```python
from build123d import *

# Parameters (mm, degrees)
SKETCH_1_W              = 510
SKETCH_1_H              = 510
EXTRUDE_1_DEPTH         = 12.5
HOLE_WIZARD_10_0_10_2_D = 10
HOLE_WIZARD_15_0_15_1_D = 15
HOLE_WIZARD_M8_1_D      = 6.8
CHAMFER_1_SIZE          = 20


with BuildPart() as part:
    # 草图1 → 凸台-拉伸1 (new, symmetric)
    with BuildSketch(Plane(origin=(0, 0, 0), x_dir=(1, 0, 0), z_dir=(0, 1, 0))):
        Rectangle(SKETCH_1_W, SKETCH_1_H)
    extrude(amount=EXTRUDE_1_DEPTH, both=True)

    # Ø10.0 (10) 直径孔2 (through all)
    with Locations(Plane(origin=(0, -12.5, 0), x_dir=(-1, 0, 0), z_dir=(0, -1, 0))):
        with Locations((188, -185), (188, -140), (-188, -185), (-188, -140), (170, 203), (125, 203), (-125, 203), (-170, 203)):
            Hole(HOLE_WIZARD_10_0_10_2_D / 2)

    # Ø15.0 (15) 直径孔1 (through all)
    with Locations(Plane(origin=(0, 12.5, 0), x_dir=(1, 0, 0), z_dir=(0, 1, 0))):
        with Locations((-240, -334.568738181), (-240, 222), (240, 222), (240, -307.647208852)):
            Hole(HOLE_WIZARD_15_0_15_1_D / 2)

    # M8 螺纹孔1 (through all)
    with Locations(Plane(origin=(0, -12.5, 0), x_dir=(-1, 0, 0), z_dir=(0, -1, 0))):
        with Locations((115, -160), (160, -160), (115, -235), (160, -235), (-160, -160), (-115, -160), (-115, -235), (-160, -235), (-235, 147), (-160, 147), (-160, 102), (-235, 102), (160, 147), (235, 147), (235, 102), (160, 102)):
            Hole(HOLE_WIZARD_M8_1_D / 2)

    # 倒角1
    chamfer_1_edges = [part.edges().sort_by_distance(p)[0] for p in [
        (-255, 0, -255),
        (255, 0, -255),
        (255, 0, 255),
        (-255, 0, 255),
    ]]
    chamfer(chamfer_1_edges, length=CHAMFER_1_SIZE)


solid = part.part
```
Geometry: final body of the model. Coordinates: model frame, mm. Coordinates: 2 decimals unless noted, no trailing zeros.
Item 1: Draft query along X for faces 1 (the face through (-4, -12.5, -4)), 2 (the face through (-245, 0, -245)), 3 (the face through (-239.024, -0.175, -229.436)), 4 (the face through (245, 0, -245)). Return one class per face: released by +X, released by -X, zero draft, split by the parting line, or undercut.
Answer:
face 1: zero draft
face 2: released by -X
face 3: undercut
face 4: released by +X
Item 2: Contact query for a flat-ended pin moving along its axis: P1, Ø5.5, axis at x = 160, z = 235, coming from the -Y side. Output: stop coordinate, or through.
Answer:
P1: passes through
Item 3: Material intervals for line 1 along X through (y, z) = (-0.5, -203); line 2 along Z through (x, y) = (188, 0); line 3 along X through (y, z) = (2.5, -102), sorted ascending.
Answer:
line 1: x = -255 to -175, -165 to -130, -120 to 120, 130 to 165, 175 to 255
line 2: z = -255 to 135, 145 to 180, 190 to 255
line 3: x = -255 to -238.4, -231.6 to -163.4, -156.6 to 156.6, 163.4 to 231.6, 238.4 to 255
